Input: part model. Units: mm. Frame: model coordinates. Face numbers are marked on the shaded views. A direction names the side the tool comes from. Coordinates: 2 decimals unless noted, no trailing zeros. Loops run counter-clockwise (first coordinate to the right, second up) from the corner with the lowest first, then second, coordinate; pieces in that order, holes last.
(1) Section A-A, the plane x = -3.5. Return loops of the section in (y, z), then the cut area to 3 significant figures.
(2) Set-up query: the marked faces 5, 6 and 7. Return all of +Z, -Z, +X, -X, +Y, -Y with unobstructed straight access to the full face (end or side cutting, diameter ignored); none if empty.
(3) Mould query, pull axis Z, two halves, no side actions, for the marked faces 1, 2, 3 and 4. Classes: released by +Z, released by -Z, zero draft, split by the parting line, or undercut.
(4) Section C-C, the plane z = 2. Return loops of the section in (x, y), then the cut area to 3 significant figures.
(5) Section D-D, the plane x = 3.25. Return loops of the section in (y, z).
(6) Contact query for flat-ended pins moving along their axis: P1, Ø5, axis at y = 12.5, z = -1.25, coming from the +X side; P2, Ø2.5, axis at x = 0, y = 20, coming from the +Z side. Output: stop coordinate, or through.
(7) Line query: L1, parallel to Y at x = 0, z = 6.6; L2, parallel to Y at x = 0.25, z = 9.25; L3, parallel to X at y = 12.5, z = 8.05. Output: solid intervals per line, ascending.
(8) Section B-B, the plane z = -2.5. Return loops of the section in (x, y).
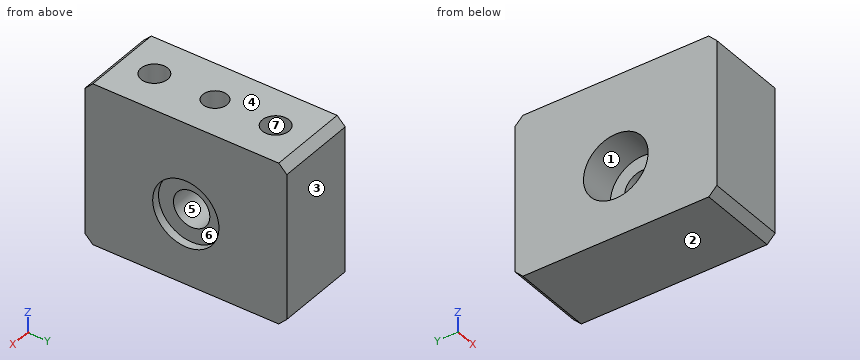
```python
from build123d import *

# Parameters (mm, degrees)
SKETCH_1_W                = 10
SKETCH_1_H                = 20
EXTRUDE_1_DEPTH           = 25
HOLE_WIZARD_1_D           = 4.5
HOLE_WIZARD_1_DEPTH       = 10.1
HOLE_WIZARD_1_CBORE_D     = 8
HOLE_WIZARD_1_CBORE_DEPTH = 4.6
HOLE_WIZARD_1_TIP         = 1.351936393
SKETCH_4_R                = 4.1
CUT_EXTRUDE_1_DEPTH       = 1
HOLE_WIZARD_M4_1_D        = 3.3
HOLE_WIZARD_M4_1_DEPTH    = 10.1
HOLE_WIZARD_M4_1_TIP      = 0.991420021
MM_1_D                    = 3
MM_1_DEPTH                = 6
MM_1_TIP                  = 0.901290929
CHAMFER_1_SIZE            = 1


with BuildPart() as part:
    # 草图1 → 凸台-拉伸1 (new body)
    with BuildSketch(Plane(origin=(0, 0, 0), x_dir=(1, 0, 0), z_dir=(0, 1, 0))):
        Rectangle(SKETCH_1_W, SKETCH_1_H)
    extrude(amount=EXTRUDE_1_DEPTH)

    # 打孔尺寸(%根据)内六角圆柱头螺钉的类型1
    with Locations(Plane.ZY.offset(5)):
        with Locations((-1.25, 12.5)):
            CounterBoreHole(HOLE_WIZARD_1_D / 2, HOLE_WIZARD_1_CBORE_D / 2, HOLE_WIZARD_1_CBORE_DEPTH, depth=HOLE_WIZARD_1_DEPTH)
            with Locations((0, 0, -(HOLE_WIZARD_1_DEPTH + HOLE_WIZARD_1_TIP / 2))):  # 118° drill point
                Cone(0, HOLE_WIZARD_1_D / 2, HOLE_WIZARD_1_TIP, mode=Mode.SUBTRACT)

    # 草图4 → 切除-拉伸1 (cut)
    with BuildSketch(Plane(origin=(5, 0, 0), x_dir=(0, 0, -1), z_dir=(1, 0, 0))):
        with Locations((1.25, 12.5)):
            Circle(SKETCH_4_R)
    extrude(amount=-CUT_EXTRUDE_1_DEPTH, mode=Mode.SUBTRACT)

    # M4 螺纹孔1
    with Locations(Plane.XY.offset(10)):
        with Locations((0, 20), (0, 5)):
            Hole(HOLE_WIZARD_M4_1_D / 2, depth=HOLE_WIZARD_M4_1_DEPTH)
            with Locations((0, 0, -(HOLE_WIZARD_M4_1_DEPTH + HOLE_WIZARD_M4_1_TIP / 2))):  # 118° drill point
                Cone(0, HOLE_WIZARD_M4_1_D / 2, HOLE_WIZARD_M4_1_TIP, mode=Mode.SUBTRACT)

    # 大小mm 暗销孔1
    with Locations(Plane.XY.offset(10)):
        with Locations((0, 12.5)):
            Hole(MM_1_D / 2, depth=MM_1_DEPTH)
            with Locations((0, 0, -(MM_1_DEPTH + MM_1_TIP / 2))):  # 118° drill point
                Cone(0, MM_1_D / 2, MM_1_TIP, mode=Mode.SUBTRACT)

    # 倒角1
    chamfer_1_edges = [part.edges().sort_by_distance(p)[0] for p in [
        (0, 25, 10),
        (0, 0, 10),
        (0, 0, -10),
        (0, 25, -10),
    ]]
    chamfer(chamfer_1_edges, length=CHAMFER_1_SIZE)


solid = part.part
```
Report:
1. outline: (0, -9) - (1, -10) - (24, -10) - (25, -9) - (25, 9) - (24, 10) - (1, 10) - (0, 9) - close; hole circle Ø8 at (12.5, -1.25)
1. area: 448 mm2
2. face 5: +X, -X
2. face 6: +X
2. face 7: +Z
3. face 1: undercut
3. face 2: released by -Z
3. face 3: zero draft
3. face 4: released by +Z
4. outline: (-5, 0) - (5, 0) - (5, 10) - (4, 10) - (4, 15) - (5, 15) - (5, 25) - (-5, 25) - (-5, 14.83) - (-0.4, 14.83) - (-0.4, 10.17) - (-5, 10.17) - close; hole circle Ø3.3 at (0, 5); hole circle Ø3.3 at (0, 20)
4. area: 206 mm2
5. outline: (0, -9) - (1, -10) - (24, -10) - (25, -9) - (25, 9) - (24, 10) - (1, 10) - (0, 9) - close; hole circle Ø4.5 at (12.5, -1.25)
6. P1: stops at x = 4
6. P2: stops at z = -0.34
7. L1: y = 0 to 3.35, 6.65 to 11, 14 to 18.35, 21.65 to 25
7. L2: y = 0.25 to 3.37, 6.63 to 11.02, 13.98 to 18.37, 21.63 to 24.75
7. L3: x = -5 to -1.5, 1.5 to 5
8. outline: (-5, 0) - (5, 0) - (5, 8.6) - (4, 8.6) - (4, 10.63) - (-0.4, 10.63) - (-0.4, 8.7) - (-5, 8.7) - close; (-5, 16.3) - (-0.4, 16.3) - (-0.4, 14.37) - (4, 14.37) - (4, 16.4) - (5, 16.4) - (5, 25) - (-5, 25) - close
